Part print with two shaded views. Sizes in mm from the minimum x, y, z corner. A direction names the side the tool comes from. Round coordinates to 2 decimals unless told otherwise and drop trailing zeros. Write each loop counter-clockwise with the first axis right and the second up, starting at its lowest first coordinate (ties: lowest second). Pieces come first, ordered by that corner, then holes. Notation, with made-up numbers: M 2.25,26.5 L 39.25,26.5 A29 ccw 39.25,54.5 Z; hole C 54.5,55 d9. An arc over 180 degrees is marked long. Use one line per item in the form item = value. Start each with the question number.
Item 1: Cut at C-C, the plane z = 27.5. Give the cut face in (x, y).
Item 2: Cut at A-A, the plane x = 6. Give the cut face in (y, z), then the cut area to 3 significant figures.
Item 3: Cut at B-B, the plane y = 9. Give the cut face in (x, z), then the cut area to 3 significant figures.
Item 4: Cut at D-D, the plane z = 7. Give the cut face in (x, y), then the cut area to 3 significant figures.
Item 5: Flat gauge pins, fed straight in: pin 1 Ø5 at (y, z) = (6.5, 31.5) entering from +X; pin 2 Ø4 at (y, z) = (9.5, 20) entering from -X; pin 3 Ø2 at (y, z) = (9, 8.5) entering from -X. Where does each tip first touch, or does it go through?
Item 6: Which spindle directions (+Z, -Z, +X, -X, +Y, -Y) get a long thin tool onto all of the face, cutting with end or side? Do the marked faces 1, 2 and 3. Say none if no direction does.
Item 7: Probe L1, parallel to Z at x = 6.25, y = 7.75; L2, parallel to Z at x = 10.25, y = 2; L3, parallel to Y at x = 10, z = 61.5 (1 decimal). List the from-to ranges inside material, lowest first.
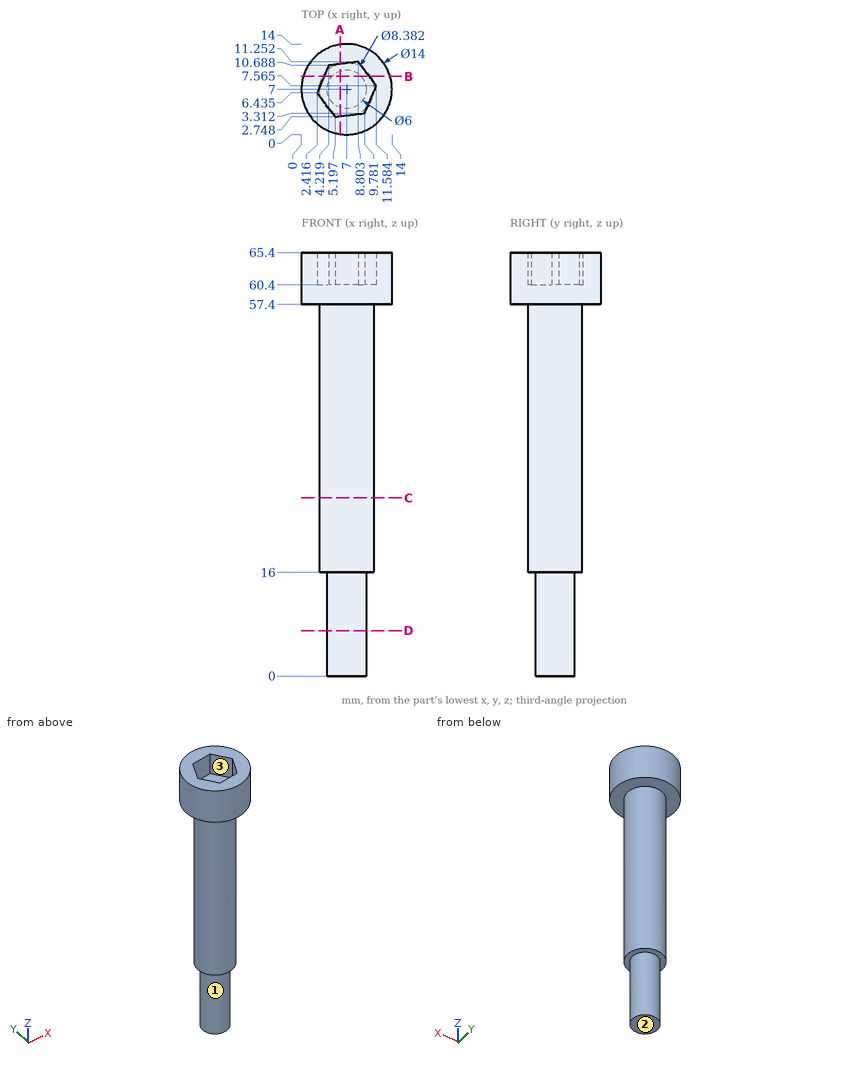
Model answer:
q1.outline = C 7,7 d8.38
q2.outline = M 0.07,57.4 L 2.93,57.4 L 2.93,16 L 4.17,16 L 4.17,0 L 9.83,0 L 9.83,16 L 11.07,16 L 11.07,57.4 L 13.93,57.4 L 13.93,65.4 L 10.91,65.4 L 10.91,60.4 L 2.85,60.4 L 2.85,65.4 L 0.07,65.4 Z
q2.area = 498 mm²
q3.outline = M 0.29,57.4 L 3.32,57.4 L 3.32,16 L 4.76,16 L 4.76,0 L 9.24,0 L 9.24,16 L 10.68,16 L 10.68,57.4 L 13.71,57.4 L 13.71,65.4 L 10.5,65.4 L 10.5,60.4 L 3.5,60.4 L 3.5,65.4 L 0.29,65.4 Z
q3.area = 449 mm²
q4.outline = C 7,7 d6
q4.area = 28.3 mm²
q5.pin_1 = 11.19
q5.pin_2 = 2.84
q5.pin_3 = 4.17
q6.face_1 = -Z
q6.face_2 = -Z, +X, -X, +Y, -Y
q6.face_3 = +Z
q7.L1 = 0 to 60.4
q7.L2 = 57.4 to 65.4
q7.L3 = 0.7 to 3.8, 9.7 to 13.3
